```python
from build123d import *

# Parameters (mm, degrees)
SKETCH_1_R          = 20
EXTRUDE_1_DEPTH     = 5
SKETCH_2_R          = 5
EXTRUDE_2_DEPTH     = 6
SKETCH_3_R          = 11.669468733
SKETCH_3_R_2        = 9.545408708
CUT_EXTRUDE_1_DEPTH = 1
SKETCH_4_R          = 1.425
EXTRUDE_3_DEPTH     = 4
SKETCH_5_R          = 17.435273898
SKETCH_5_R_2        = 15.634190673
CUT_EXTRUDE_2_DEPTH = 1
SKETCH_6_R          = 10.034081131
SKETCH_6_R_2        = 8.408881881
CUT_EXTRUDE_3_DEPTH = 1


with BuildPart() as part:
    # 草图1 → 凸台-拉伸1 (new body)
    with BuildSketch(Plane(origin=(0, 0, 0), x_dir=(1, 0, 0), z_dir=(0, 1, 0))):
        with Locations(Location((0, 0, 0), (0, 0, 270))):
            Circle(SKETCH_1_R)
    extrude(amount=EXTRUDE_1_DEPTH)

    # 草图2 → 凸台-拉伸2 (add)
    with BuildSketch(Plane.XZ):
        with Locations(Location((0, 0, 0), (0, 0, 270))):
            Circle(SKETCH_2_R)
    extrude(amount=EXTRUDE_2_DEPTH)

    # 草图3 → 切除-拉伸1 (cut)
    with BuildSketch(Plane.XZ):
        with Locations(Location((0, 0, 0), (0, 0, 270))):
            Circle(SKETCH_3_R)
        with Locations(Location((0, 0, 0), (0, 0, 270))):
            Circle(SKETCH_3_R_2, mode=Mode.SUBTRACT)
    extrude(amount=-CUT_EXTRUDE_1_DEPTH, mode=Mode.SUBTRACT)

    # 草图4 → 凸台-拉伸3 (add)
    with BuildSketch(Plane(origin=(0, 5, 0), x_dir=(1, 0, 0), z_dir=(0, 1, 0))):
        with Locations(Location((0, 0, 0), (0, 0, 270))):
            Circle(SKETCH_4_R)
    extrude(amount=EXTRUDE_3_DEPTH)

    # 草图5 → 切除-拉伸2 (cut)
    with BuildSketch(Plane(origin=(0, 5, 0), x_dir=(1, 0, 0), z_dir=(0, 1, 0))):
        with Locations(Location((0, 0, 0), (0, 0, 270))):
            Circle(SKETCH_5_R)
        with Locations(Location((0, 0, 0), (0, 0, 270))):
            Circle(SKETCH_5_R_2, mode=Mode.SUBTRACT)
    extrude(amount=-CUT_EXTRUDE_2_DEPTH, mode=Mode.SUBTRACT)

    # 草图6 → 切除-拉伸3 (cut)
    with BuildSketch(Plane(origin=(0, 5, 0), x_dir=(1, 0, 0), z_dir=(0, 1, 0))):
        with Locations(Location((0, 0, 0), (0, 0, 270))):
            Circle(SKETCH_6_R)
        with Locations(Location((0, 0, 0), (0, 0, 270))):
            Circle(SKETCH_6_R_2, mode=Mode.SUBTRACT)
    extrude(amount=-CUT_EXTRUDE_3_DEPTH, mode=Mode.SUBTRACT)


solid = part.part
```
Check sheet for the modelled part. Datum: model origin and axes. Units: mm. A direction names the side the tool comes from. Give positions to 0.01 mm unless a question says otherwise; leave off trailing zeros. Loops run counter-clockwise (first coordinate to the right, second up) from the corner with the lowest first, then second, coordinate; pieces in that order, holes last. Notation, with made-up numbers: (42, -7) - (59, -7) arc R24 ccw to (59, 23) - close; hole circle Ø8 at (-19.5, -6). An arc over 180 degrees is marked (long way). One line per question, with ' | ' between items. Start each with the question number.
1. Set-up check for faces 4 (the cylindrical face through (-10.609, 4.507, -13.836)), 5 (the cylindrical face through (11.57, 0.49, 1.52)), 6 (the cylindrical face through (-19.524, 2.465, -4.336)): record each of +Z, -Z, +X, -X, +Y, -Y from which the full face is reachable in a straight line by a thin tool's end or side.
2. Cross-section at D-D, the plane z = -5.5. Enter the section's corners in (x, y).
3. Draft check along Z on faces 1 (the flat face through (0.2, 5, 10.2)), 2 (the cylindrical face through (-4.88, -2.96, 1.08)), 3 (the flat face through (16, 4, -3)). Enter one of: released by +Z, released by -Z, zero draft, split by the parting line, or undercut.
4. Cross-section at B-B, the plane y = -2.5. Enter the section's corners in (x, z).
5. Material ranges on line 1 along X through (y, z) = (0.55, 0); line 2 along X through (y, z) = (4.35, 0); line 3 along Y through (x, z) = (-13, -4.5), recorded low to high. Write a range as [from, to].
6. Gauge pin test, flat ends, axial feed: pin 1 Ø8 at (x, z) = (-11, 9.5) entering from -Y; pin 2 Ø15.5 at (x, z) = (7, 0.5) entering from +Y; pin 3 Ø6 at (y, z) = (5.5, -6) entering from +X; pin 4 Ø4 at (x, y) = (9.5, -0.5) entering from -Z. Record the tip position at first contact, or that the pin passes through.
7. Cross-section at C-C, the plane x = -7.5. Enter the section's corners in (y, z).
Check result:
1) face 4: +Y | face 5: -Y | face 6: +Y, -Y
2) outline: (-19.23, 0) - (-10.29, 0) - (-10.29, 1) - (-7.8, 1) - (-7.8, 0) - (7.8, 0) - (7.8, 1) - (10.29, 1) - (10.29, 0) - (19.23, 0) - (19.23, 5) - (16.55, 5) - (16.55, 4) - (14.63, 4) - (14.63, 5) - (8.39, 5) - (8.39, 4) - (6.36, 4) - (6.36, 5) - (-6.36, 5) - (-6.36, 4) - (-8.39, 4) - (-8.39, 5) - (-14.63, 5) - (-14.63, 4) - (-16.55, 4) - (-16.55, 5) - (-19.23, 5) - close
3) face 1: zero draft | face 2: split by the parting line | face 3: undercut
4) outline: circle Ø10 at (0, 0)
5) line 1: x = [-20, -11.67], [-9.55, 9.55], [11.67, 20] | line 2: x = [-20, -17.44], [-15.63, -10.03], [-8.41, 8.41], [10.03, 15.63], [17.44, 20] | line 3: y = [0, 5]
6) pin 1: stops at y = 0 | pin 2: stops at y = 9 | pin 3: stops at x = 19.77 | pin 4: stops at z = -18.51
7) outline: (0, -18.54) - (5, -18.54) - (5, -15.74) - (4, -15.74) - (4, -13.72) - (5, -13.72) - (5, -6.67) - (4, -6.67) - (4, -3.8) - (5, -3.8) - (5, 3.8) - (4, 3.8) - (4, 6.67) - (5, 6.67) - (5, 13.72) - (4, 13.72) - (4, 15.74) - (5, 15.74) - (5, 18.54) - (0, 18.54) - (0, 8.94) - (1, 8.94) - (1, 5.9) - (0, 5.9) - (0, -5.9) - (1, -5.9) - (1, -8.94) - (0, -8.94) - close
